Could you check a few things on this model? Use its own coordinates, in mm. Coordinates: 2 decimals unless noted, no trailing zeros. Loops run counter-clockwise (first coordinate to the right, second up) from the corner with the lowest first, then second, coordinate; pieces in that order, holes last. Notation, with made-up numbers: M -33,-5.75 L 22,-5.75 A31 ccw 22,24.25 Z; hole C 44.25,74 d8. An arc over 180 degrees is marked long. Write each question's results on one line, items separated by ' | '.
```python
from build123d import *

# Parameters (mm, degrees)
SKETCH_1_W          = 30
SKETCH_1_H          = 30
SKETCH_1_W_2        = 24
SKETCH_1_H_2        = 24
EXTRUDE_1_DEPTH     = 940
EXTRUDE_1_2_DEPTH   = 940
EXTRUDE_1_3_DEPTH   = 940
SKETCH_3_W          = 30
SKETCH_3_H          = 30
SKETCH_3_W_2        = 24
SKETCH_3_H_2        = 24
EXTRUDE_2_DEPTH     = 480
SKETCH_4_W          = 30
SKETCH_4_H          = 480
CUT_EXTRUDE_1_DEPTH = 37
SKETCH_5_W          = 30
SKETCH_5_H          = 480
EXTRUDE_3_DEPTH     = 30
SKETCH_6_W          = 30
SKETCH_6_H          = 30
EXTRUDE_4_DEPTH     = 180


with BuildPart() as part:
    # Sketch 1 → Extrude 1 (new body)
    with BuildSketch(Plane.XY):
        with Locations((15, 15)):
            Rectangle(SKETCH_1_W, SKETCH_1_H)
        with Locations((15, 15)):
            Rectangle(SKETCH_1_W_2, SKETCH_1_H_2, mode=Mode.SUBTRACT)
    extrude(amount=EXTRUDE_1_DEPTH)



with BuildPart() as body_2:
    # Sketch 1 → Extrude 1 2 (new body)
    with BuildSketch(Plane.XY):
        with Locations((225, 15)):
            Rectangle(SKETCH_1_W, SKETCH_1_H)
        with Locations((225, 15)):
            Rectangle(SKETCH_1_W_2, SKETCH_1_H_2, mode=Mode.SUBTRACT)
    extrude(amount=EXTRUDE_1_2_DEPTH)



with BuildPart() as body_3:
    # Sketch 1 → Extrude 1 3 (new body)
    with BuildSketch(Plane.XY):
        with Locations((15, -495)):
            Rectangle(SKETCH_1_W, SKETCH_1_H)
        with Locations((15, -495)):
            Rectangle(SKETCH_1_W_2, SKETCH_1_H_2, mode=Mode.SUBTRACT)
    extrude(amount=EXTRUDE_1_3_DEPTH)


with BuildPart() as part_1:
    add(part.part)

    add(body_3.part)  # Extrude 2 merges body 3
    # Sketch 3 → Extrude 2 (add)
    with BuildSketch(Plane.XZ):
        with Locations((15, 385)):
            Rectangle(SKETCH_3_W, SKETCH_3_H)
        with Locations((15, 385)):
            Rectangle(SKETCH_3_W_2, SKETCH_3_H_2, mode=Mode.SUBTRACT)
    extrude(amount=EXTRUDE_2_DEPTH)

    # Sketch 4 → Cut-Extrude 1 (cut)
    with BuildSketch(Plane.ZY):
        with Locations((385, -240)):
            Rectangle(SKETCH_4_W, SKETCH_4_H)
    extrude(amount=-CUT_EXTRUDE_1_DEPTH, mode=Mode.SUBTRACT)


with BuildPart() as cut_extrude_1_piece_1:
    # of the separate pieces the step leaves, piece 1, a body of its own (cut_extrude_1_pieces)
    add(part_1.part.solids().sort_by_distance((0, 0, 940))[0])



with BuildPart() as cut_extrude_1_piece_2:
    # of the separate pieces the step leaves, piece 2, a body of its own (cut_extrude_1_pieces)
    add(part_1.part.solids().sort_by_distance((0, -510, 0))[0])


with BuildPart() as cut_extrude_1_piece_1_1:
    add(cut_extrude_1_piece_1.part)

    add(cut_extrude_1_piece_2.part)  # Extrude 3 merges Cut-Extrude 1 piece 2
    # Sketch 5 → Extrude 3 (add)
    with BuildSketch(Plane.ZY):
        with Locations((555, -240)):
            Rectangle(SKETCH_5_W, SKETCH_5_H)
    extrude(amount=-EXTRUDE_3_DEPTH)


with BuildPart() as body_2_1:
    add(body_2.part)

    add(cut_extrude_1_piece_1_1.part)  # Extrude 4 merges Cut-Extrude 1 piece 1
    # Sketch 6 → Extrude 4 (add)
    with BuildSketch(Plane.ZY.offset(-210)):
        with Locations((925, 15)):
            Rectangle(SKETCH_6_W, SKETCH_6_H)
    extrude(amount=EXTRUDE_4_DEPTH)


solid = body_2_1.part
```
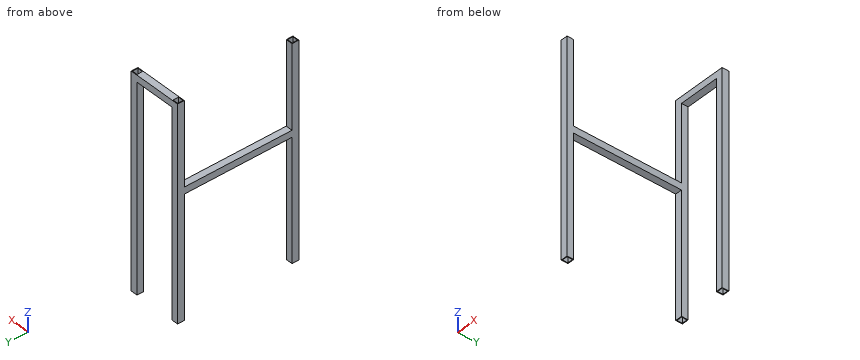
(1) Imagine slicing it at C-C, the plane y = -262. List the corners of the cut face in (x, z) for me, and give its area (3 significant figures).
Reported:
outline: M 0,540 L 30,540 L 30,570 L 0,570 Z | area: 900 mm2
(2) Will these pins go through, and if not, where does the flat tip stop? P1, Ø9, axis at y = 15, z = 560.5, coming from the -X side; P2, Ø12, axis at x = 224, z = 627, coming from the -Y side; P3, Ø24, axis at x = 9, y = -218, coming from the +Z side; P4, Ø15, axis at x = 17.5, y = -309.5, coming from the -Z side.
Reported:
P1: stops at x = 0 | P2: stops at y = 0 | P3: stops at z = 570 | P4: stops at z = 540
(3) Please list where these lines run through material, in increasing order: probe 1 along Y at (x, z) = (26.5, 237.5); probe 2 along X at (y, z) = (0.5, 760); probe 3 along Y at (x, z) = (29.5, 705). Write a range as from..to.
Reported:
probe 1: y = -510..-507, -483..-480, 0..3, 27..30 | probe 2: x = 0..30, 210..240 | probe 3: y = -510..-480, 0..30
(4) Imagine slicing it at A-A, the plane z = 103. List the corners of the cut face in (x, y) for me, and give its area (3 significant figures).
Reported:
outline: M 0,-510 L 30,-510 L 30,-480 L 0,-480 Z; M 0,0 L 30,0 L 30,30 L 0,30 Z; M 210,0 L 240,0 L 240,30 L 210,30 Z; hole M 3,-507 L 27,-507 L 27,-483 L 3,-483 Z; hole M 3,3 L 27,3 L 27,27 L 3,27 Z; hole M 213,3 L 237,3 L 237,27 L 213,27 Z | area: 972 mm2
(5) Imagine slicing it at B-B, the plane x = 53. List the corners of the cut face in (y, z) for me, and give its area (3 significant figures).
Reported:
outline: M 0,910 L 30,910 L 30,940 L 0,940 Z | area: 900 mm2
